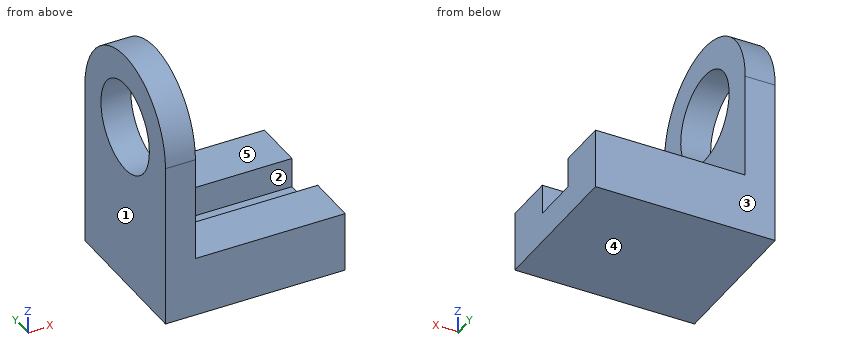
```python
from build123d import *

# Parameters (mm, degrees)
BASE_PLATE_SKETCH_W    = 60
BASE_PLATE_SKETCH_H    = 50
BASE_PLATE_DEPTH       = 10
UPRIGHT_BLOCK_SKETCH_W = 10
UPRIGHT_BLOCK_SKETCH_H = 17
UPRIGHT_BLOCK_DEPTH    = 60
BLOCK_SLOT_SKETCH_W    = 10
BLOCK_SLOT_SKETCH_H    = 50
BLOCK_SLOT_DEPTH       = 10
ROUNDED_LUG_DEPTH      = 10
LUG_HOLE_SKETCH_R      = 15
LUG_HOLE_DEPTH         = 10


with BuildPart() as part:
    # Base Plate Sketch → Base Plate (new body)
    with BuildSketch(Plane.XY):
        with Locations((30, 25)):
            Rectangle(BASE_PLATE_SKETCH_W, BASE_PLATE_SKETCH_H)
    extrude(amount=BASE_PLATE_DEPTH)

    # Upright Block Sketch → Upright Block (add)
    with BuildSketch(Plane(origin=(60, 0, 0), x_dir=(0, 0, -1), z_dir=(1, 0, 0))):
        with Locations((-15, 41.5)):
            Rectangle(UPRIGHT_BLOCK_SKETCH_W, UPRIGHT_BLOCK_SKETCH_H)
        with Locations((-15, 8.5)):
            Rectangle(UPRIGHT_BLOCK_SKETCH_W, UPRIGHT_BLOCK_SKETCH_H)
    extrude(amount=-UPRIGHT_BLOCK_DEPTH)

    # Block Slot Sketch → Block Slot (cut)
    with BuildSketch(Plane.XY.offset(20)):
        with Locations((5, 25)):
            Rectangle(BLOCK_SLOT_SKETCH_W, BLOCK_SLOT_SKETCH_H)
    extrude(amount=-BLOCK_SLOT_DEPTH, mode=Mode.SUBTRACT)

    # Rounded Lug Sketch → Rounded Lug (add)
    with BuildSketch(Plane.ZY):
        with BuildLine():
            Line((20, 50), (10, 50))
            Line((10, 50), (10, 0))
            Line((10, 0), (20, 0))
            Line((20, 0), (55, 0))
            ThreePointArc((55, 0), (80, 25), (55, 50))
            Line((55, 50), (20, 50))
        make_face()
    extrude(amount=-ROUNDED_LUG_DEPTH)

    # Lug Hole Sketch → Lug Hole (cut)
    with BuildSketch(Plane(origin=(10, 0, 0), x_dir=(0, 0, -1), z_dir=(1, 0, 0))):
        with Locations((-55, 25)):
            Circle(LUG_HOLE_SKETCH_R)
    extrude(amount=-LUG_HOLE_DEPTH, mode=Mode.SUBTRACT)


solid = part.part
```
Can you work these out from the model? Positions are in its coordinate system, mm. Face numbers are marked on the shaded views. A direction names the side the tool comes from. Coordinates: 2 decimals unless noted, no trailing zeros. Loops run counter-clockwise (first coordinate to the right, second up) from the corner with the lowest first, then second, coordinate; pieces in that order, holes last. Notation, with made-up numbers: (40, 89.5) -> (54, 89.5) arc R26 ccw to (54, 108.5) -> close; hole circle Ø7 at (-13, -36). An arc over 180 degrees is marked (long way). Put each result on its own line as item: value. Start each with the question number.
Q1. If I drill on line 1 (Y direction, x = 51, z = 18); line 2 (Y direction, x = 5.75, z = 55); line 3 (Z direction, x = 14.5, y = 46), over which ranges is the centre line in solid material (lowest first)? Write a range as [from, to].
Q2. I want a section at C-C (z = 62). Write out the boundary of the cut face in (x, y), plus the area to 3 significant figures.
Q3. I want a section at A-A (y = 25). Write out the boundary of the cut face in (x, z), plus the area to 3 significant figures.
Q4. For the marked faces 4 and 5, which set-ups out of +Z, -Z, +X, -X, +Y, -Y let a thin tool reach every point of the face, with its end or its side?
Q5. I want a section at D-D (y = 32). Write out the boundary of the cut face in (x, z), plus the area to 3 significant figures.
Q6. I want a section at B-B (x = 5). Write out the boundary of the cut face in (y, z), plus the area to 3 significant figures.
Q7. Thinking about a two-plate mould opening in Y: for the marked faces 1, 2 and 3, which applies, pulls with the +Y half, pulls with the -Y half, needs draft (parallel to the pull), parting line crosses it, or undercut?
Q8. I'm going to push flat-ended pins straight in: P1, Ø6, axis at x = 23, y = 15.5, coming from the +Z side; P2, Ø25, axis at y = 33.5, z = 62, coming from the +X side; P3, Ø4, axis at x = 8.5, y = 7.5, coming from the +Z side. Where does each tip first touch, or does it pass through?
Taken from the geometry:
1. line 1: y = [0, 17], [33, 50]
1. line 2: y = [0, 10], [40, 50]
1. line 3: z = [0, 20]
2. outline: (0, 1) -> (10, 1) -> (10, 11.73) -> (0, 11.73) -> close; (0, 38.27) -> (10, 38.27) -> (10, 49) -> (0, 49) -> close
2. area: 215 mm2
3. outline: (0, 0) -> (60, 0) -> (60, 10) -> (10, 10) -> (10, 40) -> (0, 40) -> close; (0, 70) -> (10, 70) -> (10, 80) -> (0, 80) -> close
3. area: 1,000 mm2
4. face 4: -Z, +X, -X, +Y, -Y
4. face 5: +Z, +X, +Y, -Y
5. outline: (0, 0) -> (60, 0) -> (60, 10) -> (10, 10) -> (10, 41.73) -> (0, 41.73) -> close; (0, 68.27) -> (10, 68.27) -> (10, 79) -> (0, 79) -> close
5. area: 1,020 mm2
6. outline: (0, 0) -> (50, 0) -> (50, 55) arc R25 ccw to (0, 55) -> close; hole circle Ø30 at (25, 55)
6. area: 3,020 mm2
7. face 1: needs draft
7. face 2: undercut
7. face 3: pulls with the +Y half
8. P1: stops at z = 20
8. P2: stops at x = 10
8. P3: stops at z = 74.62
